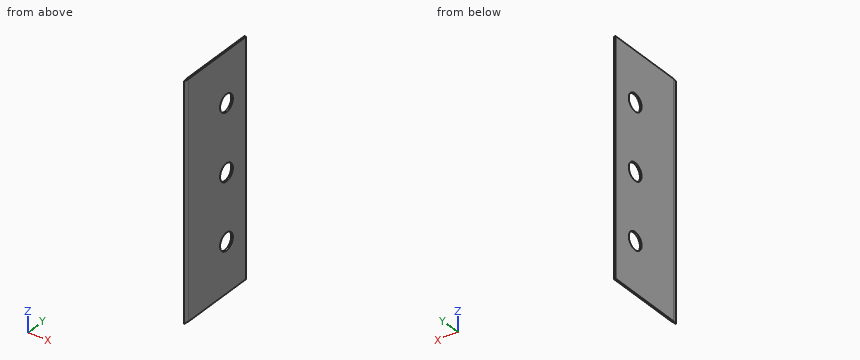
```python
from build123d import *

# Parameters (mm, degrees)
SKETCH_1_W                  = 70
SKETCH_1_H                  = 25
EXTRUDE_1_DEPTH             = 0.5
CUT_EXTRUDE_1_DEPTH         = 72.109071151
HOLE_WIZARD_5_2_5_2_1_D     = 5.2
HOLE_WIZARD_5_2_5_2_1_DEPTH = 19.75
HOLE_WIZARD_5_2_5_2_1_TIP   = 1.562237609


with BuildPart() as part:
    # 草图1 → 凸台-拉伸1 (new body)
    with BuildSketch(Plane(origin=(0, 0, 0), x_dir=(0, 0, -1), z_dir=(1, 0, 0))):
        Rectangle(SKETCH_1_W, SKETCH_1_H)
    extrude(amount=EXTRUDE_1_DEPTH)

    # 草图2 → 切除-拉伸1 (cut, through all)
    with BuildSketch(Plane.XY.offset(35)):
        Polygon((0.25, -12.5), (0, -11), (-1.209013091, -11.201502182), (-0.510365148, -13.117899248), (1.363353431, -13.117899248), (1.198992152, -10.8497136), (0.5, -11), align=None)
    extrude(amount=-CUT_EXTRUDE_1_DEPTH, mode=Mode.SUBTRACT)

    # Ø5.2 (5.2) 直径孔1
    with Locations(Plane.ZY):
        with Locations((-20, 4.5), (0, 4.5), (20, 4.5)):
            Hole(HOLE_WIZARD_5_2_5_2_1_D / 2, depth=HOLE_WIZARD_5_2_5_2_1_DEPTH)
            with Locations((0, 0, -(HOLE_WIZARD_5_2_5_2_1_DEPTH + HOLE_WIZARD_5_2_5_2_1_TIP / 2))):  # 118° drill point
                Cone(0, HOLE_WIZARD_5_2_5_2_1_D / 2, HOLE_WIZARD_5_2_5_2_1_TIP, mode=Mode.SUBTRACT)


solid = part.part
```
Check sheet for the modelled part. Datum: model origin and axes. Units: mm. Coordinates: 2 decimals unless noted, no trailing zeros. Order: outer loops, then holes, each group sorted by start corner. A loop starts at its lowest first (then second) coordinate and runs counter-clockwise, first axis right, second up. Notation, with made-up numbers: (16, 68.5) -> (25, 68.5) arc R18 cw to (25, 97.5) -> close; hole circle Ø1 at (-28, 73.25). An arc over 180 degrees is marked (long way). Write item = value, one per line. Start each with the question number.
1) Cross-section at A-A (y = 4.5). Enter the section's corners in (x, z), then the cut area to 3 significant figures.
2) Cross-section at B-B (z = 0). Enter the section's corners in (x, y), then the cut area to 4 significant figures.
3) Cross-section at D-D (z = 16). Enter the section's corners in (x, y).
4) Material ranges on L1, parallel to Z at x = 0.3, y = 3.5; L2, parallel to Z at x = 0.4, y = 3.25, recorded low to high.
5) Cross-section at C-C (x = 0.15). Enter the section's corners in (y, z).
Ans:
q1.outline = (0, -35) -> (0.5, -35) -> (0.5, -22.6) -> (0, -22.6) -> close; (0, -17.4) -> (0.5, -17.4) -> (0.5, -2.6) -> (0, -2.6) -> close; (0, 2.6) -> (0.5, 2.6) -> (0.5, 17.4) -> (0, 17.4) -> close; (0, 22.6) -> (0.5, 22.6) -> (0.5, 35) -> (0, 35) -> close
q1.area = 27.2 mm²
q2.outline = (0, -11) -> (0.25, -12.5) -> (0.5, -11) -> (0.5, 1.9) -> (0, 1.9) -> close; (0, 7.1) -> (0.5, 7.1) -> (0.5, 12.5) -> (0, 12.5) -> close
q2.area = 9.525 mm²
q3.outline = (0, -11) -> (0.25, -12.5) -> (0.5, -11) -> (0.5, 12.5) -> (0, 12.5) -> close
q4.L1 = -35 to -22.4, -17.6 to -2.4, 2.4 to 17.6, 22.4 to 35
q4.L2 = -35 to -22.28, -17.72 to -2.28, 2.28 to 17.72, 22.28 to 35
q5.outline = (-11.9, -35) -> (12.5, -35) -> (12.5, 35) -> (-11.9, 35) -> close; hole circle Ø5.2 at (4.5, -20); hole circle Ø5.2 at (4.5, 0); hole circle Ø5.2 at (4.5, 20)
